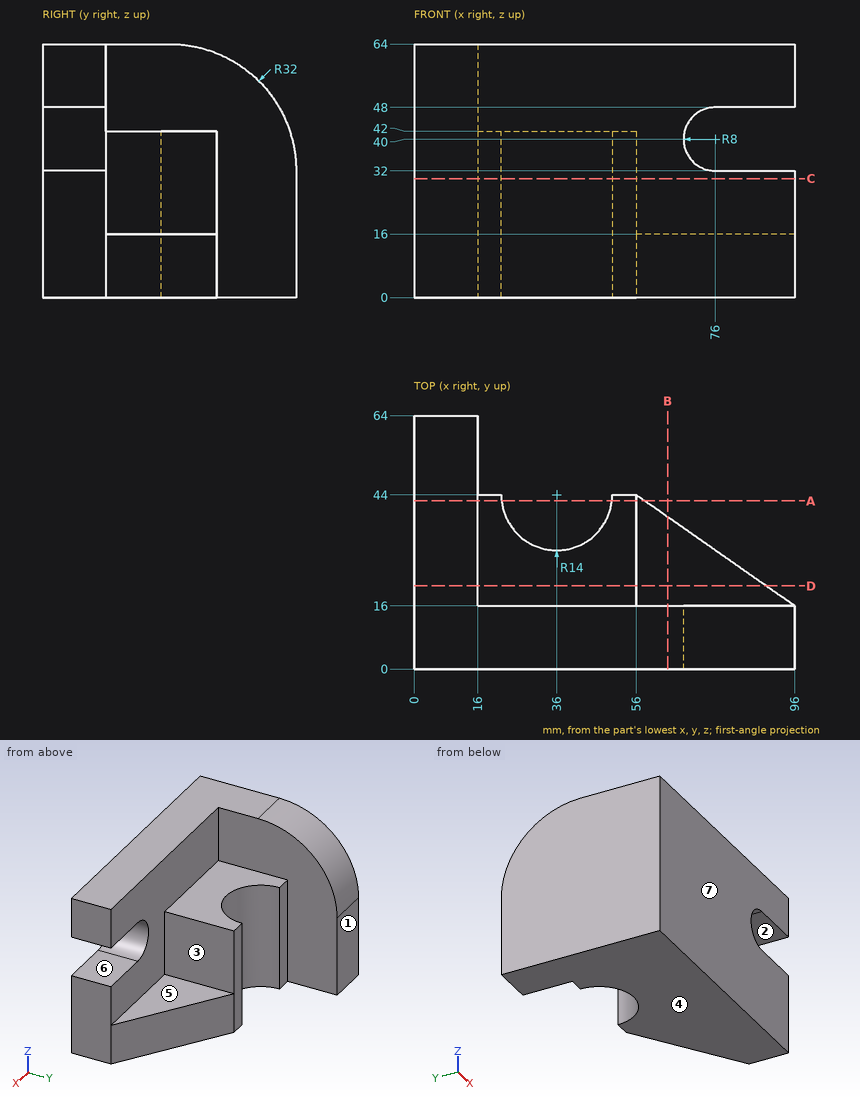
Part print with two shaded views. Sizes in mm from the minimum x, y, z corner. A direction names the side the tool comes from. Coordinates: 2 decimals unless noted, no trailing zeros. Loops run counter-clockwise (first coordinate to the right, second up) from the corner with the lowest first, then second, coordinate; pieces in that order, holes last. Notation, with made-up numbers: (41, 72.5) -> (71, 72.5) arc R19 cw to (71, 93.5) -> close; hole circle Ø1 at (76, 83.5). An arc over 180 degrees is marked (long way). Answer as a JSON object with one key per item and string values.
Q1. Cut at A-A (y = 42.5). List the corners of the cut face in (x, z), and give its area (3 significant figures).
Report:
{"outline": "(0, 0) -> (22.08, 0) -> (22.08, 42) -> (16, 42) -> (16, 62.23) -> (0, 62.23) -> close; (49.92, 0) -> (58.14, 0) -> (58.14, 16) -> (56, 16) -> (56, 42) -> (49.92, 42) -> close", "area": "1,540 mm2"}
Q2. Flat gauge pins, fed straight in: P1, Ø4, axis at x = 64, y = 34, coming from the +Z side; P2, Ø8, axis at y = 35.5, z = 30, coming from the +X side; P3, Ø22.5, axis at x = 39.5, y = 30.5, coming from the +Z side; P4, Ø2, axis at x = 76, z = 33.5, coming from the +Y side. Where does each tip first touch, or does it go through?
Report:
{"P1": "stops at z = 16", "P2": "stops at x = 56", "P3": "stops at z = 42", "P4": "passes through"}
Q3. Pull direction Z, two halves, no side cores. Call the marked faces 4, 5, 6 and 7: released by +Z, released by -Z, zero draft, split by the parting line, or undercut.
Report:
{"face 4": "released by -Z", "face 5": "released by +Z", "face 6": "undercut", "face 7": "zero draft"}
Q4. Cut at C-C (z = 30). List the corners of the cut face in (x, y).
Report:
{"outline": "(0, 0) -> (96, 0) -> (96, 16) -> (56, 16) -> (56, 44) -> (50, 44) arc R14 cw to (22, 44) -> (16, 44) -> (16, 64) -> (0, 64) -> close"}
Q5. 3-axis set-ups, long thin cutter, end or side, ignore diameter. For the marked faces 1, 2 and 3: which of +Z, -Z, +X, -X, +Y, -Y reach the whole face in a straight line?
Report:
{"face 1": "+Z, -Z, +X, -X, +Y", "face 2": "+X, +Y, -Y", "face 3": "+Z, +X, +Y"}
Q6. Cut at D-D (y = 21). List the corners of the cut face in (x, z).
Report:
{"outline": "(0, 0) -> (88.86, 0) -> (88.86, 16) -> (56, 16) -> (56, 42) -> (16, 42) -> (16, 64) -> (0, 64) -> close"}
Q7. Probe probe 1 along X at (y, z) = (56.5, 35.5); probe 2 along Y at (x, z) = (20, 34). List the from-to ranges inside material, lowest first.
Report:
{"probe 1": "x = 0 to 16", "probe 2": "y = 0 to 44"}
Q8. Cut at B-B (x = 64). List the corners of the cut face in (y, z).
Report:
{"outline": "(0, 0) -> (38.4, 0) -> (38.4, 16) -> (16, 16) -> (16, 64) -> (0, 64) -> close"}
